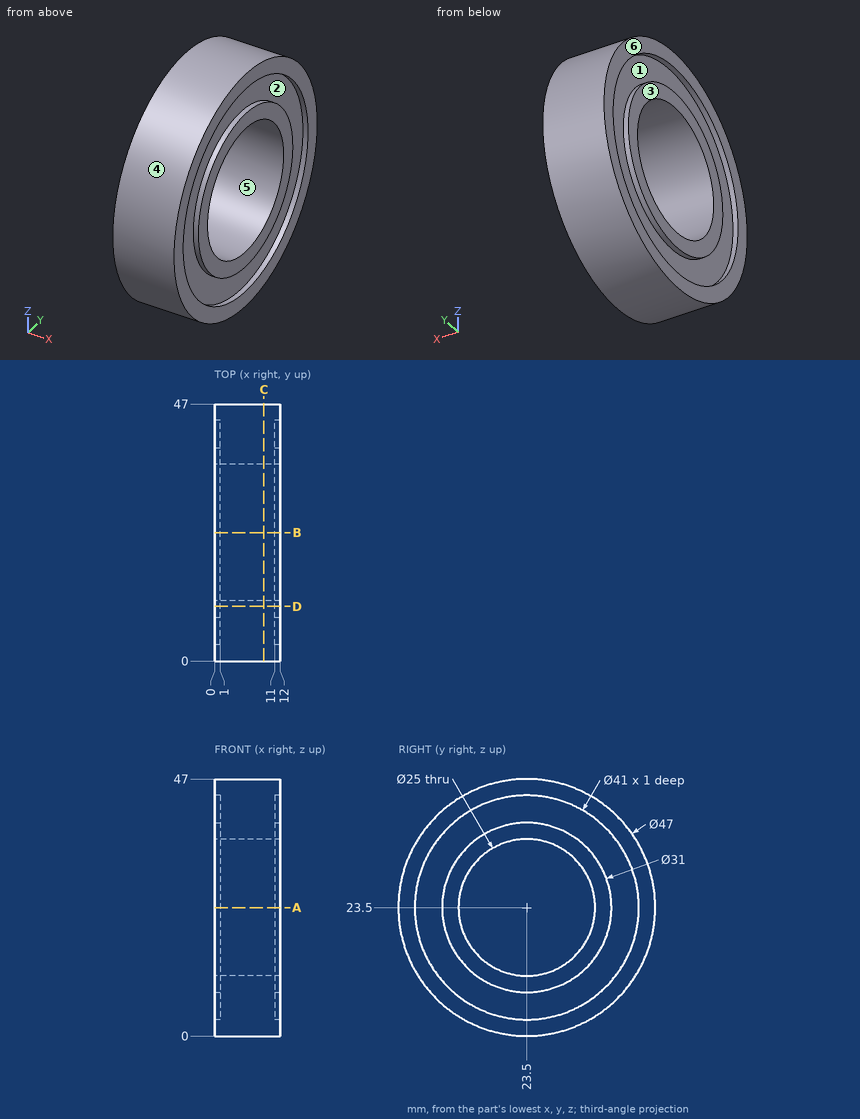
Design review of the part shown in the three views and the two pictorial views. Dimensions are in mm from the part's minimum x, y and z. A direction names the side the tool comes from. Coordinates: 2 decimals unless noted, no trailing zeros. Order: outer loops, then holes, each group sorted by start corner. A loop starts at its lowest first (then second) coordinate and runs counter-clockwise, first axis right, second up.
1) Wall thickness on line 1 along Y through (x, z) = (0.35, 23.5); line 2 along Y through (x, z) = (7, 23.5); line 3 along Y through (x, z) = (8, 13.5): over which ranges is each line inside the solid? List them lowest first.
2) Take a section at D-D, the plane y = 10. Give the boundary of the cut face in (x, z).
3) For the marked faces 1, 2 and 3, list the 3-axis set-ups (+Z, -Z, +X, -X, +Y, -Y) from which the entire face can be reached by the end or side of a thin tool; tool diameter is ignored.
4) Clearance check with flat-ended pins moving along their axes: pin 1 (5 mm diameter, centred on x = 1.5, z = 12.5, fed in from +Y); pin 2 (1 mm diameter, centred on x = 1.5, y = 12, fed in from -Z); pin 3 (22.5 mm diameter, centred on y = 23.5, z = 23.5, fed in from -X); pin 4 (6 mm diameter, centred on x = 1, z = 29, fed in from +Y). State where each tip first meets the part, or that it passes through.
5) Take a section at C-C, the plane x = 9. Give the boundary of the cut face in (y, z).
6) Take a section at A-A, the plane z = 23.5. Give the boundary of the cut face in (x, y), and give its area (3 significant figures).
7) Mouldability with a two-part tool opening along Z and no side actions: class the marked faces 4, 5 and 6 as +Z half, -Z half, draft (parallel to the pull), parting line (faces both ways), or undercut.
Returned:
1. line 1: y = 0 to 3, 8 to 11, 36 to 39, 44 to 47
1. line 2: y = 0 to 11, 36 to 47
1. line 3: y = 2.23 to 16, 31 to 44.77
2. outline: (0, 4.26) - (12, 4.26) - (12, 8.07) - (11, 8.07) - (11, 15.88) - (12, 15.88) - (12, 31.12) - (11, 31.12) - (11, 38.93) - (12, 38.93) - (12, 42.74) - (0, 42.74) - (0, 38.93) - (1, 38.93) - (1, 31.12) - (0, 31.12) - (0, 15.88) - (1, 15.88) - (1, 8.07) - (0, 8.07) - close
3. face 1: -X
3. face 2: +X
3. face 3: +Z, -Z, -X, +Y, -Y
4. pin 1: stops at y = 45.41
4. pin 2: stops at z = 2.73
4. pin 3: passes through
4. pin 4: stops at y = 46.87
5. outline: circle Ø47 at (23.5, 23.5); hole circle Ø25 at (23.5, 23.5)
6. outline: (0, 0) - (12, 0) - (12, 3) - (11, 3) - (11, 8) - (12, 8) - (12, 11) - (0, 11) - (0, 8) - (1, 8) - (1, 3) - (0, 3) - close; (0, 36) - (12, 36) - (12, 39) - (11, 39) - (11, 44) - (12, 44) - (12, 47) - (0, 47) - (0, 44) - (1, 44) - (1, 39) - (0, 39) - close
6. area: 244 mm2
7. face 4: parting line
7. face 5: undercut
7. face 6: draft
